Source: CAD feature listing. Evaluate the final solid. Frame: model axes, mm. Give positions to 0.01 mm unless a question says otherwise; leave off trailing zeros. Loops run counter-clockwise (first coordinate to the right, second up) from the corner with the lowest first, then second, coordinate; pieces in that order, holes last. Notation, with made-up numbers: (-12.75, -17) - (6.25, -17) arc R14 cw to (6.25, -3) - close; hole circle Ø6 at (33.5, -39.5). An arc over 180 degrees is marked (long way). Put each result on its own line as item: value.
```python
from build123d import *

# Parameters (mm, degrees)
FILLET1_R = 1.5


with BuildPart() as part:
    # Sketch1 → Revolve1 (revolve)
    with BuildSketch(Plane.XY, mode=Mode.PRIVATE) as revolve1_sk:
        with BuildLine():
            Line((5.120546846, 31.7), (12.5, 31.7))
            Line((12.5, 31.7), (12.5, 22.5))
            Line((12.5, 22.5), (-12.5, 22.5))
            Line((-12.5, 22.5), (-12.5, 31.7))
            Line((-12.5, 31.7), (-5.120546846, 31.7))
            ThreePointArc((-5.120546846, 31.7), (0, 29.4), (5.120546846, 31.7))
        make_face()
    revolve(revolve1_sk.sketch.rotate(Axis((-18.919268053, 0, 0), (1, 0, 0)), 90), axis=Axis((-18.919268053, 0, 0), (1, 0, 0)))

    # Fillet1
    fillet1_edges = [part.edges().sort_by_distance(p)[0] for p in [
        (12.5, 0, -22.5),
        (-12.5, 0, -22.5),
    ]]
    fillet(fillet1_edges, radius=FILLET1_R)


solid = part.part
```
1) Section query C-C, the plane x = 0. Output: boundary loops of the cut face in (y, z), plus the area to 3 significant figures.
Check result:
outline: circle Ø58.8 at (0, 0); hole circle Ø45 at (0, 0)
area: 1,130 mm²
2) Pin query (flat end, axial travel): P1, Ø1, axis at x = 4.5, y = -21, coming from the +Z side; P2, Ø10, axis at y = -2.5, z = -15.5, coming from the +X side; P3, Ø4, axis at x = 1.5, y = -7.5, coming from the +Z side; P4, Ø12, axis at x = 6.5, z = -3, coming from the -Y side. Return the tip coordinate at first contact, or that it passes through.
Check result:
P1: z = 23.7
P2: through
P3: z = 29.52
P4: y = -31.7
3) Mould query, pull axis Z, two halves, no side actions, for faces 1 (the cylindrical face through (-0.154, 19.961, 10.382)), 2 (the flat face through (-12.5, -24, 5)), 3 (the cylindrical face through (-8.76, -31.43, -4.13)). Classes: pulls with the +Z half, pulls with the -Z half, needs draft (parallel to the pull), parting line crosses it, or undercut.
Check result:
face 1: undercut
face 2: needs draft
face 3: parting line crosses it
4) Section query A-A, the plane y = 0. Output: boundary loops of the cut face in (x, z).
Check result:
outline: (-12.5, -31.7) - (-5.12, -31.7) arc R6.85 cw to (5.12, -31.7) - (12.5, -31.7) - (12.5, -24) arc R1.5 ccw to (11, -22.5) - (-11, -22.5) arc R1.5 ccw to (-12.5, -24) - close; (-12.5, 24) arc R1.5 ccw to (-11, 22.5) - (11, 22.5) arc R1.5 ccw to (12.5, 24) - (12.5, 31.7) - (5.12, 31.7) arc R6.85 cw to (-5.12, 31.7) - (-12.5, 31.7) - close
5) Material intervals for line 1 along Y through (x, z) = (5.25, 0); line 2 along Y through (x, z) = (-10.75, 2.5); line 3 along Z through (x, y) = (-11.25, -13), sorted ascending. Write a range as [from, to].
Check result:
line 1: [-31.7, -22.5], [22.5, 31.7]
line 2: [-31.6, -22.36], [22.36, 31.6]
line 3: [-28.91, -18.39], [18.39, 28.91]
6) Section query D-D, the plane x = -8.25. Output: boundary loops of the cut face in (y, z).
Check result:
outline: circle Ø63.4 at (0, 0); hole circle Ø45 at (0, 0)
